Geometry check sheet. Reference: the model listing, model coordinates, mm. Give positions to 0.01 mm unless a question says otherwise; leave off trailing zeros. Loops run counter-clockwise (first coordinate to the right, second up) from the corner with the lowest first, then second, coordinate; pieces in that order, holes last. Notation, with made-up numbers: (59, 40) -> (103, 40) arc R18 ccw to (103, 46) -> close; hole circle Ø2 at (-19.5, 54.5). An arc over 180 degrees is marked (long way). One line per item, written item: value. Start each with the question number.
(1) Sectioned sample at A-A, the plane x = 263.5. Record the cut outline in (y, z), then the cut area to 3 significant figures.
(2) Gauge pin test, flat ends, axial feed: pin 1 Ø8 at (x, y) = (-394, -30) entering from +Z; pin 2 Ø10 at (x, y) = (590, 50) entering from -Z; pin 3 Ø7.5 at (x, y) = (-546.5, 20) entering from +Z. Record the tip position at first contact, or that the pin passes through.
(3) Scan lines: line 1 along Y through (x, z) = (-394, 2.5); line 2 along Y through (x, z) = (590, 5.75); line 3 along Z through (x, y) = (311, -3.5). Record each from-to range of solid material in increasing order. Write a range as from..to.
from build123d import *

# Parameters (mm, degrees)
SKETCH_1_W                  = 1200
SKETCH_1_H                  = 120
EXTRUDE_1_DEPTH             = 7.5
HOLE_WIZARD_3_D             = 6.6
HOLE_WIZARD_3_CBORE_D       = 11
HOLE_WIZARD_3_CBORE_DEPTH   = 6.8
HOLE_WIZARD_3_2_D           = 9
HOLE_WIZARD_3_2_CBORE_D     = 15
HOLE_WIZARD_3_2_CBORE_DEPTH = 9
SKETCH_7_W                  = 2
SKETCH_7_H                  = 15.2
CUT_EXTRUDE_1_DEPTH         = 1202.5224717


with BuildPart() as part:
    # 草图1 → 凸台-拉伸1 (new, symmetric)
    with BuildSketch(Plane.XY):
        Rectangle(SKETCH_1_W, SKETCH_1_H)
    extrude(amount=EXTRUDE_1_DEPTH, both=True)

    # Hole Wizard 3 (through all)
    with Locations(Plane(origin=(590, 50, -7.5), x_dir=(-1, 0, 0), z_dir=(0, 0, -1))):
        with Locations((0, 0)):
            CounterBoreHole(HOLE_WIZARD_3_D / 2, HOLE_WIZARD_3_CBORE_D / 2, HOLE_WIZARD_3_CBORE_DEPTH)

    # Hole Wizard 3 2 (through all)
    with Locations(Plane(origin=(-550, 20, 7.5), x_dir=(1, 0, 0), z_dir=(0, 0, 1))):
        with Locations((0, 0), (156, 0), (156, -50), (0, -50)):
            CounterBoreHole(HOLE_WIZARD_3_2_D / 2, HOLE_WIZARD_3_2_CBORE_D / 2, HOLE_WIZARD_3_2_CBORE_DEPTH)

    # 草图7 → 切除-拉伸1 (cut, through all)
    with BuildSketch(Plane(origin=(600, 0, 0), x_dir=(0, 0, -1), z_dir=(1, 0, 0))):
        with Locations((-6.5, -2.4)):
            Rectangle(SKETCH_7_W, SKETCH_7_H)
    extrude(amount=-CUT_EXTRUDE_1_DEPTH, mode=Mode.SUBTRACT)


solid = part.part
Calculated:
1. outline: (-60, -7.5) -> (60, -7.5) -> (60, 7.5) -> (5.2, 7.5) -> (5.2, 5.5) -> (-10, 5.5) -> (-10, 7.5) -> (-60, 7.5) -> close
1. area: 1,770 mm2
2. pin 1: passes through
2. pin 2: stops at z = -0.7
2. pin 3: stops at z = -1.5
3. line 1: y = -60..-37.5, -22.5..12.5, 27.5..60
3. line 2: y = -60..-10, 5.2..46.7, 53.3..60
3. line 3: z = -7.5..5.5
